The listing builds one solid part. Answer for the finished solid, in the listing's coordinates (mm). A direction names the side the tool comes from. Coordinates: 2 decimals unless noted, no trailing zeros. Write each loop counter-clockwise with the first axis right and the second up, starting at its lowest first coordinate (ties: lowest second). Pieces come first, ordered by that corner, then holes.
(1) The part is cut by section C-C on y = 7. Determine the outline of the cut face in (x, z), plus the area to 3 significant figures.
(2) Straight lines are drawn through the part: line 1 (Y direction, x = 5.75, z = 5); line 2 (Y direction, x = 4.75, z = 5); line 3 (Y direction, x = -7.5, z = 4.25). For each, find the intervals that lie inside material, in ascending order.
(3) The part is cut by section B-B on x = 1. Determine the outline of the cut face in (y, z).
(4) For a pull along Y with two mould halves and no side action, classify faces 1 (the cylindrical face through (-1.19, -1.63, 3.35)), 2 (the flat face through (5, 15, 10)), 3 (the flat face through (0, 7, 10)) as +Y half, -Y half, draft (parallel to the pull), parting line (faces both ways), or undercut.
(5) The part is cut by section A-A on z = 5. Determine the outline of the cut face in (x, y).
(6) The part is cut by section D-D on x = 5. Determine the outline of the cut face in (y, z).
(7) Given P1, Ø5, axis at y = 6.5, z = 8, coming from the -X side; P2, Ø3, axis at x = -4.5, z = 7.5, coming from the +Y side, each flat-ended and moving along its own axis, determine where each tip first touches the part or whether it passes through.
(8) Which of the six approach directions +Z, -Z, +X, -X, +Y, -Y give full straight-line access (tool end or side, diameter ignored) to faces 4 (the flat face through (-5, 0, 10)), 5 (the flat face through (0, -15, 10)), 6 (the flat face through (4, -7, 6.8))?
from build123d import *

# Parameters (mm, degrees)
SKETCH_1_W                = 20
SKETCH_1_H                = 30
EXTRUDE_1_DEPTH           = 20
HOLE_WIZARD_1_D           = 6.6
HOLE_WIZARD_1_CBORE_D     = 11
HOLE_WIZARD_1_CBORE_DEPTH = 6.8
SKETCH_4_W                = 10
SKETCH_4_H                = 15
CUT_EXTRUDE_1_DEPTH       = 27.925824036
HOLE_WIZARD_M4_1_D        = 3.3
CHAMFER_1_SIZE            = 0.5


with BuildPart() as part:
    # 草图1 → 凸台-拉伸1 (new body)
    with BuildSketch(Plane.XY):
        Rectangle(SKETCH_1_W, SKETCH_1_H)
    extrude(amount=EXTRUDE_1_DEPTH)

    # 打孔尺寸根据内六角圆柱头螺钉的类型1 (through all)
    with Locations(Plane(origin=(3.133596483, 10.907898158, 0), x_dir=(1, 0, 0), z_dir=(0, 0, -1))):
        with Locations((-3.133596483, 17.907898158)):
            CounterBoreHole(HOLE_WIZARD_1_D / 2, HOLE_WIZARD_1_CBORE_D / 2, HOLE_WIZARD_1_CBORE_DEPTH)

    # 草图4 → 切除-拉伸1 (cut, through all)
    with BuildSketch(Plane.XY.offset(20)):
        with Locations((-5, 7.5)):
            Rectangle(SKETCH_4_W, SKETCH_4_H)
    extrude(amount=-CUT_EXTRUDE_1_DEPTH, mode=Mode.SUBTRACT)

    # M4 螺纹孔1 (through all)
    with Locations(Plane.ZY):
        with Locations((5, 7)):
            Hole(HOLE_WIZARD_M4_1_D / 2)

    # 倒角1
    chamfer_1_edges = [part.edges().sort_by_distance(p)[0] for p in [
        (-10, 0, 10),
        (0, 15, 10),
        (10, -15, 10),
        (-10, -15, 10),
        (10, 15, 10),
    ]]
    chamfer(chamfer_1_edges, length=CHAMFER_1_SIZE)


solid = part.part
Model answer:
1. outline: (0, 0) - (10, 0) - (10, 3.35) - (0, 3.35) - close; (0, 6.65) - (10, 6.65) - (10, 20) - (0, 20) - close
1. area: 167 mm2
2. line 1: y = -15 to 5.35, 8.65 to 15
2. line 2: y = -15 to -9.77, -4.23 to 5.35, 8.65 to 15
2. line 3: y = -15 to 0
3. outline: (-15, 0) - (-12.41, 0) - (-12.41, 6.8) - (-10.14, 6.8) - (-10.14, 20) - (-15, 20) - close; (-3.86, 6.8) - (-1.59, 6.8) - (-1.59, 0) - (15, 0) - (15, 20) - (-3.86, 20) - close; hole circle Ø3.3 at (7, 5)
4. face 1: undercut
4. face 2: +Y half
4. face 3: draft
5. outline: (-10, -14.5) - (-9.5, -15) - (9.5, -15) - (10, -14.5) - (10, 5.35) - (0, 5.35) - (0, 0) - (-9.5, 0) - (-10, -0.5) - close; (0, 8.65) - (10, 8.65) - (10, 14.5) - (9.5, 15) - (0.5, 15) - (0, 14.5) - close; hole circle Ø11 at (0, -7)
6. outline: (-15, 0) - (-9.29, 0) - (-9.29, 6.8) - (-4.71, 6.8) - (-4.71, 0) - (15, 0) - (15, 20) - (-15, 20) - close; hole circle Ø3.3 at (7, 5)
7. P1: stops at x = 0
7. P2: stops at y = 0
8. face 4: +Z, -Z, -X, +Y
8. face 5: +Z, -Z, +X, -X, -Y
8. face 6: -Z
